Design review of the part built by this model. Coordinates are the model's own, in mm. Face numbers are marked on the shaded views. A direction names the side the tool comes from. Coordinates: 2 decimals unless noted, no trailing zeros. Loops run counter-clockwise (first coordinate to the right, second up) from the corner with the lowest first, then second, coordinate; pieces in that order, holes last.
Q1. Add section A-A on y = 0. Give the boundary of the cut face in (x, z), and give its area (4 significant figures).
Q2. Add section B-B on x = 5. Give the boundary of the cut face in (y, z).
Q3. Add section C-C on z = -5.75. Give the boundary of the cut face in (x, y), and give its area (3 significant figures).
Q4. Draft analysis for pull direction Y (two halves, no side actions). For the marked faces 1, 2 and 3, state which applies: released by +Y, released by -Y, zero draft, split by the parting line, or undercut.
Q5. Add section D-D on x = 0. Give the boundary of the cut face in (y, z).
Q6. Wall thickness on probe 1 along Y at (x, z) = (0, 1.75); probe 2 along Y at (x, z) = (0, -4); probe 3 along Y at (x, z) = (4, 4): over which ranges is each line inside the solid? List them lowest first.
Q7. For P1, Ø2, axis at x = -2.5, y = 4.5, coming from the +Z side; P2, Ø5, axis at x = 1, y = 2, coming from the -Z side; P3, Ø2.5, axis at x = 0, y = 0.5, coming from the -Z side, all flat-tipped, find the tip position at first contact; note any pin that passes through.
Q8. Machinability: for the marked faces 4, 5 and 6, which of the approach directions +Z, -Z, +X, -X, +Y, -Y give a long, thin tool a straight path to every point of the face, cutting with its end or side? Answer none if there is none.
```python
from build123d import *

# Parameters (mm, degrees)
SKETCH_1_R           = 8
EXTRUDE_1_DEPTH      = 7.5
SKETCH_3_R           = 2.5
CUT_EXTRUDE_2_DEPTH  = 12.5
SKETCH_4_OUTSIDE_W   = 23.43
SKETCH_4_OUTSIDE_H   = 23.43
SKETCH_4_OUTSIDE_W_2 = 12
SKETCH_4_OUTSIDE_H_2 = 20.092263618
CUT_EXTRUDE_3_DEPTH  = 19.788294228
SKETCH_5_W           = 16.185662541
SKETCH_5_H           = 6.325725708
CUT_EXTRUDE_4_DEPTH  = 19.027756377
SKETCH_8_W           = 12
SKETCH_8_H           = 2.708497378
EXTRUDE_2_DEPTH      = 15
CHAMFER_1_SIZE       = 0.5
SKETCH_2_W           = 17
SKETCH_2_H           = 3
CUT_EXTRUDE_5_DEPTH  = 6
CHAMFER_2_SIZE       = 0.5


with BuildPart() as part:
    # 草图1 → 凸台-拉伸1 (new, symmetric)
    with BuildSketch(Plane.XY):
        Circle(SKETCH_1_R)
    extrude(amount=EXTRUDE_1_DEPTH, both=True)

    # 草图3 → 切除-拉伸2 (cut)
    with BuildSketch(Plane(origin=(0, 0, -7.5), x_dir=(-1, 0, 0), z_dir=(0, 0, -1))):
        Circle(SKETCH_3_R)
    extrude(amount=-CUT_EXTRUDE_2_DEPTH, mode=Mode.SUBTRACT)

    # 草图4 outside → 切除-拉伸3 (cut, through all)
    with BuildSketch(Plane.XY.offset(7.5)):
        Rectangle(SKETCH_4_OUTSIDE_W, SKETCH_4_OUTSIDE_H)
        Rectangle(SKETCH_4_OUTSIDE_W_2, SKETCH_4_OUTSIDE_H_2, mode=Mode.SUBTRACT)
    extrude(amount=-CUT_EXTRUDE_3_DEPTH, mode=Mode.SUBTRACT)

    # 草图5 → 切除-拉伸4 (cut, through all)
    with BuildSketch(Plane.XY.offset(7.5)):
        with Locations((0.239490277, -6.162862854)):
            Rectangle(SKETCH_5_W, SKETCH_5_H)
    extrude(amount=-CUT_EXTRUDE_4_DEPTH, mode=Mode.SUBTRACT)

    # 草图8 → 凸台-拉伸2 (add)
    with BuildSketch(Plane(origin=(0, 0, -7.5), x_dir=(-1, 0, 0), z_dir=(0, 0, -1))):
        with Locations((0, 6.645751311)):
            Rectangle(SKETCH_8_W, SKETCH_8_H)
    extrude(amount=-EXTRUDE_2_DEPTH)

    # 倒角1
    chamfer_1_edges = [part.edges().sort_by_distance(p)[0] for p in [
        (6, -3, 0),
        (-6, -3, 0),
        (6, 8, 0),
        (-6, 8, 0),
    ]]
    chamfer(chamfer_1_edges, length=CHAMFER_1_SIZE)

    # 草图2 → 切除-拉伸5 (cut)
    with BuildSketch(Plane.XY.offset(7.5)):
        with Locations((0.206171625, 4.7)):
            Rectangle(SKETCH_2_W, SKETCH_2_H)
    extrude(amount=-CUT_EXTRUDE_5_DEPTH, mode=Mode.SUBTRACT)

    # 倒角2
    chamfer_2_edges = [part.edges().sort_by_distance(p)[0] for p in [
        (6, 3.2, 4.5),
        (6, 6.2, 4.5),
        (-6, 6.2, 4.5),
        (-6, 3.2, 4.5),
        (0, 3.2, 7.5),
    ]]
    chamfer(chamfer_2_edges, length=CHAMFER_2_SIZE)


solid = part.part
```
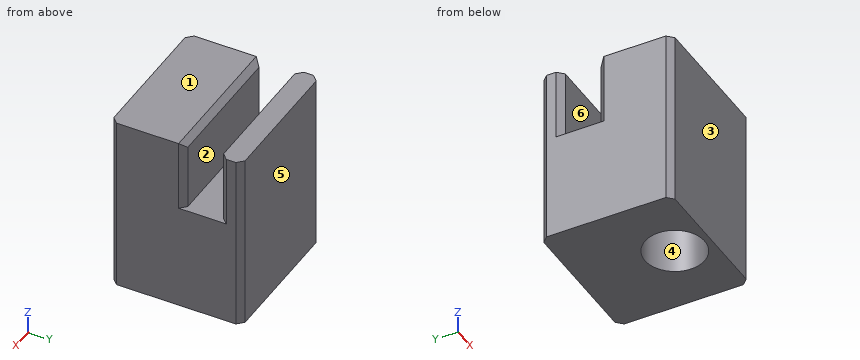
Entries:
1. outline: (-6, -7.5) - (-2.5, -7.5) - (-2.5, 5) - (2.5, 5) - (2.5, -7.5) - (6, -7.5) - (6, 7.5) - (-6, 7.5) - close
1. area: 117.5 mm2
2. outline: (-3, -7.5) - (8, -7.5) - (8, 7.5) - (6.2, 7.5) - (6.2, 1.5) - (3.2, 1.5) - (3.2, 7) - (2.7, 7.5) - (-3, 7.5) - close
3. outline: (-6, -2.5) - (-5.5, -3) - (5.5, -3) - (6, -2.5) - (6, 7.5) - (5.5, 8) - (-5.5, 8) - (-6, 7.5) - close; hole circle Ø5 at (0, 0)
3. area: 112 mm2
4. face 1: zero draft
4. face 2: undercut
4. face 3: released by -Y
5. outline: (-3, -7.5) - (-2.5, -7.5) - (-2.5, 5) - (2.5, 5) - (2.5, -7.5) - (8, -7.5) - (8, 7.5) - (6.2, 7.5) - (6.2, 1.5) - (3.2, 1.5) - (3.2, 7) - (2.7, 7.5) - (-3, 7.5) - close
6. probe 1: y = -3 to -2.5, 2.5 to 3.2, 6.2 to 8
6. probe 2: y = -3 to -2.5, 2.5 to 8
6. probe 3: y = -3 to 3.2, 6.2 to 8
7. P1: stops at z = 1.5
7. P2: stops at z = -7.5
7. P3: stops at z = 5
8. face 4: -Z
8. face 5: +Z, -Z, +X, -X, +Y
8. face 6: +Z, +X, -X
